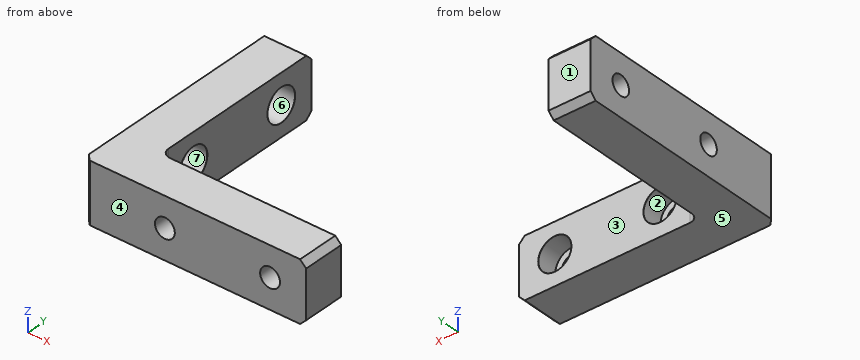
```python
from build123d import *

# Parameters (mm, degrees)
EXTRUDE_1_DEPTH          = 10
FILLET_1_R               = 3
CHAMFER_1_SIZE           = 2
CHAMFER_2_SIZE           = 2
HOLE_WIZARD_1_AT_2_COUNT = 2
HOLE_WIZARD_1_AT_2_PITCH = 35
HOLE_WIZARD_2_AT_2_COUNT = 2
HOLE_WIZARD_2_AT_2_PITCH = 35


with BuildPart() as part:
    # 草图1 → 凸台-拉伸1 (new, symmetric)
    with BuildSketch(Plane.XY):
        Polygon((0, 0), (-74, 0), (-74, 74), (-60, 74), (-60, 14), (0, 14), align=None)
    extrude(amount=EXTRUDE_1_DEPTH, both=True)

    # 圆角1
    fillet_1_edges = [part.edges().sort_by_distance(p)[0] for p in [
        (-60, 14, 0),
    ]]
    fillet(fillet_1_edges, radius=FILLET_1_R)

    # 倒角1
    chamfer_1_edges = [part.edges().sort_by_distance(p)[0] for p in [
        (-67, 74, 10),
        (0, 7, 10),
        (-67, 74, -10),
        (0, 7, -10),
    ]]
    chamfer(chamfer_1_edges, length=CHAMFER_1_SIZE)

    # 倒角2
    chamfer_2_edges = [part.edges().sort_by_distance(p)[0] for p in [
        (-74, 0, 0),
    ]]
    chamfer(chamfer_2_edges, length=CHAMFER_2_SIZE)

    # 草图2 → 打孔尺寸(%根据)内六角圆柱头螺钉的类型1 (revolve, cut)
    with BuildSketch(Plane(origin=(-60, 62, 0), x_dir=(0, 0, -1), z_dir=(0, 1, 0))):
        Polygon((0, 0), (0, 14), (3.3, 14), (3.3, 6.8), (5.5, 6.8), (5.5, 0.025), (5.525, 0), align=None)
    hole_wizard_1 = revolve(axis=Axis((-53.65, 62, 0), (-1, 0, 0)), mode=Mode.SUBTRACT)

    # 打孔尺寸(%根据)内六角圆柱头螺钉的类型1 at 2: 打孔尺寸(%根据)内六角圆柱头螺钉的类型1 ×2
    with Locations(*[(0, -i * HOLE_WIZARD_1_AT_2_PITCH, 0) for i in range(1, HOLE_WIZARD_1_AT_2_COUNT)]):
        add(hole_wizard_1, mode=Mode.SUBTRACT)

    # 草图4 → 打孔尺寸(%根据)内六角圆柱头螺钉的类型2 (revolve, cut)
    with BuildSketch(Plane(origin=(-12, 14, 0), x_dir=(0, 0, 1), z_dir=(1, 0, 0))):
        Polygon((0, 0), (0, 14), (3.3, 14), (3.3, 6.8), (5.5, 6.8), (5.5, 0.025), (5.525, 0), align=None)
    hole_wizard_2 = revolve(axis=Axis((-12, 20.35, 0), (0, -1, 0)), mode=Mode.SUBTRACT)

    # 打孔尺寸(%根据)内六角圆柱头螺钉的类型2 at 2: 打孔尺寸(%根据)内六角圆柱头螺钉的类型2 ×2
    with Locations(*[(-i * HOLE_WIZARD_2_AT_2_PITCH, 0, 0) for i in range(1, HOLE_WIZARD_2_AT_2_COUNT)]):
        add(hole_wizard_2, mode=Mode.SUBTRACT)


solid = part.part
```
Input: part model. Units: mm. Frame: model coordinates. Face numbers are marked on the shaded views. A direction names the side the tool comes from. Give positions to 0.01 mm unless a question says otherwise; leave off trailing zeros. Order: outer loops, then holes, each group sorted by start corner. A loop starts at its lowest first (then second) coordinate and runs counter-clockwise, first axis right, second up. Notation, with made-up numbers: M -11.5,87.25 L 47.5,87.25 A16 ccw 47.5,111.25 Z; hole C 74,-15.5 d6. An arc over 180 degrees is marked long. One line per question, with ' | ' between items. Start each with the question number.
1. Section query D-D (z = 0). Count the separate pieces of the cut face and the enclosed holes in it, and give its area (3 significant figures).
2. Pull-direction query (Y, two-part tool) for the marked faces 4, 5, 6 and 7; classes: released by +Y, released by -Y, zero draft, split by the parting line, or undercut.
3. Section query A-A (y = 62). Return the cut outline in (x, z) (3 decimals), and give its area (3 significant figures).
4. Section query B-B (x = -47). Return the cut outline in (y, z) (3 decimals), and give its area (3 significant figures).
5. First-contact query: pin 1 Ø12 at (y, z) = (26.5, -2.5) entering from +X; pin 2 Ø5.5 at (x, z) = (-49, 2.5) entering from +Y; pin 3 Ø5.5 at (x, z) = (-12, -1.5) entering from +Y. Flat tips, straight axial feed; report the tip coordinate or a pass-through.
6. Access query for the marked faces 1, 2 and 3. Directions: +Z, -Z, +X, -X, +Y, -Y. A direction counts if a zero-diameter tool reaches every point of the face in a straight line with its end or side. Return the directions, or none.
7. Material intervals for probe 1 along X at (y, z) = (2.75, 0); probe 2 along Y at (x, z) = (-62.5, 0); probe 3 along Y at (x, z) = (-71.5, 0), sorted ascending. Write a range as [from, to].
8. Section query C-C (x = -65). Return the cut outline in (y, z), and give its area (3 significant figures).
Here are the results:
1) separate pieces: 5 | enclosed holes: 0 | area: 1,390 mm²
2) face 4: released by -Y | face 5: zero draft | face 6: undercut | face 7: undercut
3) outline: M -74,-10 L -60,-10 L -60,-5.525 L -60.025,-5.5 L -66.8,-5.5 L -66.8,-3.3 L -74,-3.3 Z; M -74,3.3 L -66.8,3.3 L -66.8,5.5 L -60.025,5.5 L -60,5.525 L -60,10 L -74,10 Z | area: 158 mm²
4) outline: M 0,-10 L 14,-10 L 14,-5.525 L 13.975,-5.5 L 7.2,-5.5 L 7.2,-3.3 L 0,-3.3 Z; M 0,3.3 L 7.2,3.3 L 7.2,5.5 L 13.975,5.5 L 14,5.525 L 14,10 L 0,10 Z | area: 158 mm²
5) pin 1: x = -60 | pin 2: y = 14 | pin 3: y = 7.2
6) face 1: +Z, -Z, +X, -X, +Y | face 2: +Y | face 3: +Z, -Z, +X, +Y
7) probe 1: [-74, -50.3], [-43.7, -15.3], [-8.7, 0] | probe 2: [0, 21.5], [32.5, 56.5], [67.5, 74] | probe 3: [0, 23.7], [30.3, 58.7], [65.3, 74]
8) outline: M 0,-10 L 72,-10 L 74,-8 L 74,8 L 72,10 L 0,10 Z; hole C 27,0 d11; hole C 62,0 d11 | area: 1,290 mm²
